The listing builds one solid part. Answer for the finished solid, in the listing's coordinates (mm). A direction names the side the tool comes from. Coordinates: 2 decimals unless noted, no trailing zeros. Order: outer loops, then holes, each group sorted by start corner. A loop starts at its lowest first (then second) coordinate and runs counter-clockwise, first axis right, second up. Notation, with made-up numbers: M 71,58.5 L 81,58.5 A20 ccw 81,70.5 Z; hole C 60,-29 d2. An arc over 180 degrees is marked long. One line per item, written item: value. Start each with the question number.
Q1. Each of these flat-tipped pins is pushed along its axis until it touches: pin 1 Ø6 at (y, z) = (-29.5, 96) entering from +X; pin 2 Ø6 at (x, z) = (124.77, 20) entering from -Y; pin 3 Ø8.5 at (x, z) = (284.77, 140) entering from +Y; pin 4 Ø8 at (y, z) = (-13.5, 124.5) entering from -X. Where does it stop, or does it pass through?
Q2. For faces 4 (the flat face through (44.81, -21.61, 78.88)), 5 (the flat face through (39.111, -27.386, 78.88)), determine the directions among +Z, -Z, +X, -X, +Y, -Y from which every point of the face is accessible in a straight line to the end or side of a thin tool.
Q3. Determine the mould class of faces 1 (the conical face through (281.212, -52.67, 140.157)), 2 (the flat face through (227, -49.358, 79)), 3 (the flat face through (185, -51, 0)) for opening direction Z: pulls with the +Z half, pulls with the -Z half, needs draft (parallel to the pull), parting line crosses it, or undercut.
Q4. Straight lines are drawn through the part: line 1 along X through (y, z) = (-50, 20); line 2 along X through (y, z) = (-50.6, 140); line 3 along Y through (x, z) = (293, 58). For each, find the intervals that lie inside material, in ascending order. Write a range as [from, to].
Q5. The part is cut by section B-B on x = 257. Give the vertices of the cut face in (y, z).
Q6. The part is cut by section C-C on y = -16. Give the vertices of the cut face in (x, z).
Q7. The part is cut by section A-A on z = 43. Give the vertices of the cut face in (x, y).
```python
from build123d import *

# Parameters (mm, degrees)
BOSS_EXTRUDE4_DEPTH          = 160
SKETCH24_R                   = 3.25
CUT_EXTRUDE3_DEPTH           = 8
SKETCH26_R                   = 8.25
CUT_EXTRUDE4_DEPTH           = 5
CUT_EXTRUDE4_DRAFT           = -45
CUT_EXTRUDE4_PROFILE_2_DEPTH = 5
CUT_EXTRUDE4_PROFILE_2_DRAFT = -45
CUT_EXTRUDE4_PROFILE_3_DEPTH = 5
CUT_EXTRUDE4_PROFILE_3_DRAFT = -45
CUT_EXTRUDE4_PROFILE_4_DEPTH = 5
CUT_EXTRUDE4_PROFILE_4_DRAFT = -45
FILLET1_R                    = 10
FILLET2_R                    = 2


with BuildPart() as part:
    # Sketch23 → Boss-Extrude4 (new body)
    with BuildSketch(Plane.XY):
        Polygon((4.588611491, 6.553216354), (0, 0), (81.915204429, -57.357643635), (366.915204429, -57.357643635), (401.55622058, -37.357643635), (397.55622058, -30.429440405), (364.771610889, -49.357643635), (84.43759474, -49.357643635), align=None)
    extrude(amount=BOSS_EXTRUDE4_DEPTH)

    # Sketch24 → Cut-Extrude3 (cut)
    with BuildSketch(Plane(origin=(0, -49.357643635, 0), x_dir=(1, 0, 0), z_dir=(0, 1, 0))):
        with Locations(Location((124.771610889, -20, 0), (0, 0, 270))):
            Circle(SKETCH24_R)
        with Locations(Location((284.771610889, -20, 0), (0, 0, 270))):
            Circle(SKETCH24_R)
        with Locations(Location((124.771610889, -140, 0), (0, 0, 270))):
            Circle(SKETCH24_R)
        with Locations(Location((284.771610889, -140, 0), (0, 0, 270))):
            Circle(SKETCH24_R)
    extrude(amount=-CUT_EXTRUDE3_DEPTH, mode=Mode.SUBTRACT)


with BuildPart() as cut_extrude4_tool:
    # Sketch26 → Cut-Extrude4 (with draft: the straight prism first)
    with BuildSketch(Plane.XZ.offset(57.357643635)):
        with Locations((124.771610889, 140)):
            Circle(SKETCH26_R)
    extrude(amount=-CUT_EXTRUDE4_DEPTH)
    # Cut-Extrude4: the draft: its side faces are tilted about the plane it starts from
    cut_extrude4_sides = [cut_extrude4_tool.faces().sort_by_distance(p)[0] for p in [
        (116.521610889, -54.857643635, 140),
    ]]
    draft(cut_extrude4_sides, Plane.XZ.offset(57.357643635), CUT_EXTRUDE4_DRAFT)


with BuildPart() as part_1:
    add(part.part)

    # Cut-Extrude4: cut by cut_extrude4_tool
    add(cut_extrude4_tool.part, mode=Mode.SUBTRACT)


with BuildPart() as cut_extrude4_profile_2_tool:
    # Sketch26 → Cut-Extrude4 profile 2 (with draft: the straight prism first)
    with BuildSketch(Plane.XZ.offset(57.357643635)):
        with Locations((284.771610889, 140)):
            Circle(SKETCH26_R)
    extrude(amount=-CUT_EXTRUDE4_PROFILE_2_DEPTH)
    # Cut-Extrude4 profile 2: the draft: its side faces are tilted about the plane it starts from
    cut_extrude4_profile_2_sides = [cut_extrude4_profile_2_tool.faces().sort_by_distance(p)[0] for p in [
        (276.521610889, -54.857643635, 140),
    ]]
    draft(cut_extrude4_profile_2_sides, Plane.XZ.offset(57.357643635), CUT_EXTRUDE4_PROFILE_2_DRAFT)


with BuildPart() as part_2:
    add(part_1.part)

    # Cut-Extrude4 profile 2: cut by cut_extrude4_profile_2_tool
    add(cut_extrude4_profile_2_tool.part, mode=Mode.SUBTRACT)


with BuildPart() as cut_extrude4_profile_3_tool:
    # Sketch26 → Cut-Extrude4 profile 3 (with draft: the straight prism first)
    with BuildSketch(Plane.XZ.offset(57.357643635)):
        with Locations((284.771610889, 20)):
            Circle(SKETCH26_R)
    extrude(amount=-CUT_EXTRUDE4_PROFILE_3_DEPTH)
    # Cut-Extrude4 profile 3: the draft: its side faces are tilted about the plane it starts from
    cut_extrude4_profile_3_sides = [cut_extrude4_profile_3_tool.faces().sort_by_distance(p)[0] for p in [
        (276.521610889, -54.857643635, 20),
    ]]
    draft(cut_extrude4_profile_3_sides, Plane.XZ.offset(57.357643635), CUT_EXTRUDE4_PROFILE_3_DRAFT)


with BuildPart() as part_3:
    add(part_2.part)

    # Cut-Extrude4 profile 3: cut by cut_extrude4_profile_3_tool
    add(cut_extrude4_profile_3_tool.part, mode=Mode.SUBTRACT)


with BuildPart() as cut_extrude4_profile_4_tool:
    # Sketch26 → Cut-Extrude4 profile 4 (with draft: the straight prism first)
    with BuildSketch(Plane.XZ.offset(57.357643635)):
        with Locations((124.771610889, 20)):
            Circle(SKETCH26_R)
    extrude(amount=-CUT_EXTRUDE4_PROFILE_4_DEPTH)
    # Cut-Extrude4 profile 4: the draft: its side faces are tilted about the plane it starts from
    cut_extrude4_profile_4_sides = [cut_extrude4_profile_4_tool.faces().sort_by_distance(p)[0] for p in [
        (116.521610889, -54.857643635, 20),
    ]]
    draft(cut_extrude4_profile_4_sides, Plane.XZ.offset(57.357643635), CUT_EXTRUDE4_PROFILE_4_DRAFT)


with BuildPart() as part_4:
    add(part_3.part)

    # Cut-Extrude4 profile 4: cut by cut_extrude4_profile_4_tool
    add(cut_extrude4_profile_4_tool.part, mode=Mode.SUBTRACT)

    # Fillet1
    fillet1_edges = [part_4.edges().sort_by_distance(p)[0] for p in [
        (366.915204429, -57.357643635, 80),
        (81.915204429, -57.357643635, 80),
    ]]
    fillet(fillet1_edges, radius=FILLET1_R)

    # Fillet2
    fillet2_edges = [part_4.edges().sort_by_distance(p)[0] for p in [
        (84.43759474, -49.357643635, 80),
        (364.771610889, -49.357643635, 80),
    ]]
    fillet(fillet2_edges, radius=FILLET2_R)


solid = part_4.part
```
Output:
1. pin 1: stops at x = 398.75
1. pin 2: passes through
1. pin 3: stops at y = -49.36
1. pin 4: stops at x = 13.57
2. face 4: +Z, -Z, +Y
2. face 5: +Z, -Z, -X, -Y
3. face 1: undercut
3. face 2: needs draft
3. face 3: pulls with the -Z half
4. line 1: x = [71.41, 121.52], [128.02, 281.52], [288.02, 379.66]
4. line 2: x = [72.26, 121.52], [128.02, 281.52], [288.02, 378.62]
4. line 3: y = [-57.36, -49.36]
5. outline: M -57.36,0 L -49.36,0 L -49.36,160 L -57.36,160 Z
6. outline: M 22.85,0 L 36.8,0 L 36.8,160 L 22.85,160 Z
7. outline: M 0,0 L 79.33,-55.55 A10 ccw 85.07,-57.36 L 364.24,-57.36 A10 ccw 369.24,-56.02 L 401.56,-37.36 L 397.56,-30.43 L 365.24,-49.09 A2 cw 364.24,-49.36 L 85.07,-49.36 A2 cw 83.92,-49 L 4.59,6.55 Z
